Source: CAD feature listing. Evaluate the final solid. Frame: model axes, mm. Round coordinates to 2 decimals unless told otherwise and drop trailing zeros. Write each loop counter-clockwise with the first axis right and the second up, starting at its lowest first coordinate (ties: lowest second). Pieces come first, ordered by that corner, then holes. Notation, with made-up numbers: M 14,4 L 18,4 A24 ccw 18,31 Z; hole C 30,4.5 d10. An arc over 180 degrees is marked long. Answer in a Markdown table with one row per item. Add a question column.
Item 1: Contact query for a flat-ended pin moving along its axis: pin 1 (10 mm diameter, centred on x = 634.5, z = 7, fed in from -Y). Output: stop coordinate, or through.
Item 2: Material intervals for probe 1 along X at (y, z) = (-75, 18), sorted ascending.
Item 3: Cut plane B-B on y = -72. Return loops of the section in (x, z).
Item 4: Cut plane A-A on z = 15.25. Return loops of the section in (x, y), and give its area (3 significant figures).
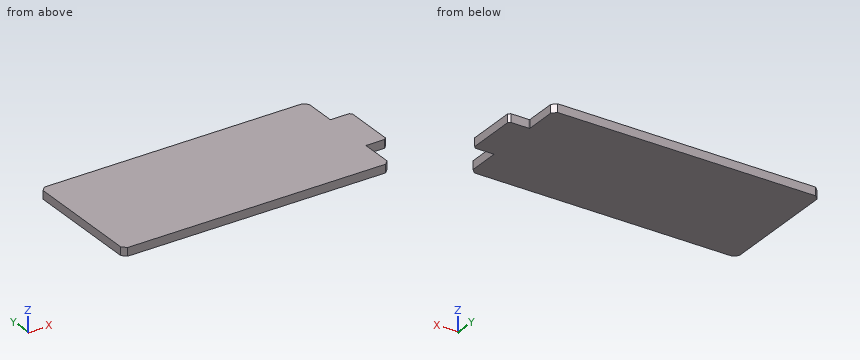
from build123d import *

# Parameters (mm, degrees)
BOSS_EXTRUDE1_DEPTH = 20
CHAMFER1_SIZE       = 10
FILLET1_R           = 1
CHAMFER2_SIZE       = 5


with BuildPart() as part:
    # Sketch1 → Boss-Extrude1 (new body)
    with BuildSketch(Plane.XY):
        Polygon((-38.770663033, -150), (-38.770663033, 150), (601.229336967, 150), (601.229336967, 64), (651.229336967, 64), (651.229336967, -64), (601.229336967, -64), (601.229336967, -150), align=None)
    extrude(amount=BOSS_EXTRUDE1_DEPTH)

    # Chamfer1
    chamfer1_edges = [part.edges().sort_by_distance(p)[0] for p in [
        (601.229336967, 150, 10),
        (601.229336967, -150, 10),
        (-38.770663033, -150, 10),
        (-38.770663033, 150, 10),
    ]]
    chamfer(chamfer1_edges, length=CHAMFER1_SIZE)

    # Fillet1
    fillet1_edges = [part.edges().sort_by_distance(p)[0] for p in [
        (601.229336967, 64, 10),
        (601.229336967, -64, 10),
    ]]
    fillet(fillet1_edges, radius=FILLET1_R)

    # Chamfer2
    chamfer2_edges = [part.edges().sort_by_distance(p)[0] for p in [
        (651.229336967, 64, 10),
        (651.229336967, -64, 10),
    ]]
    chamfer(chamfer2_edges, length=CHAMFER2_SIZE)


solid = part.part
Results below:
| question | item | result |
|---|---|---|
| 1 | pin 1 | y = -64 |
| 2 | probe 1 | -38.77 to 601.23 |
| 3 | outline | M -38.77,0 L 601.23,0 L 601.23,20 L -38.77,20 Z |
| 4 | outline | M -38.77,-140 L -28.77,-150 L 591.23,-150 L 601.23,-140 L 601.23,-65 A1 cw 602.23,-64 L 646.23,-64 L 651.23,-59 L 651.23,59 L 646.23,64 L 602.23,64 A1 cw 601.23,65 L 601.23,140 L 591.23,150 L -28.77,150 L -38.77,140 Z |
| 4 | area | 198,000 mm2 |
